Print and shaded views of the part. All mm, measured from the part's lowest x, y and z. A direction names the side the tool comes from. Round coordinates to 2 decimals unless told otherwise and drop trailing zeros. Write each loop counter-clockwise with the first axis right and the second up, starting at its lowest first coordinate (ties: lowest second). Pieces come first, ordered by that corner, then holes. Notation, with made-up numbers: M -34,-26 L -28,-26 A8 cw -28,-17 Z; hole C 16.25,-38 d8. An arc over 180 degrees is marked long. Write item = value, one per line.
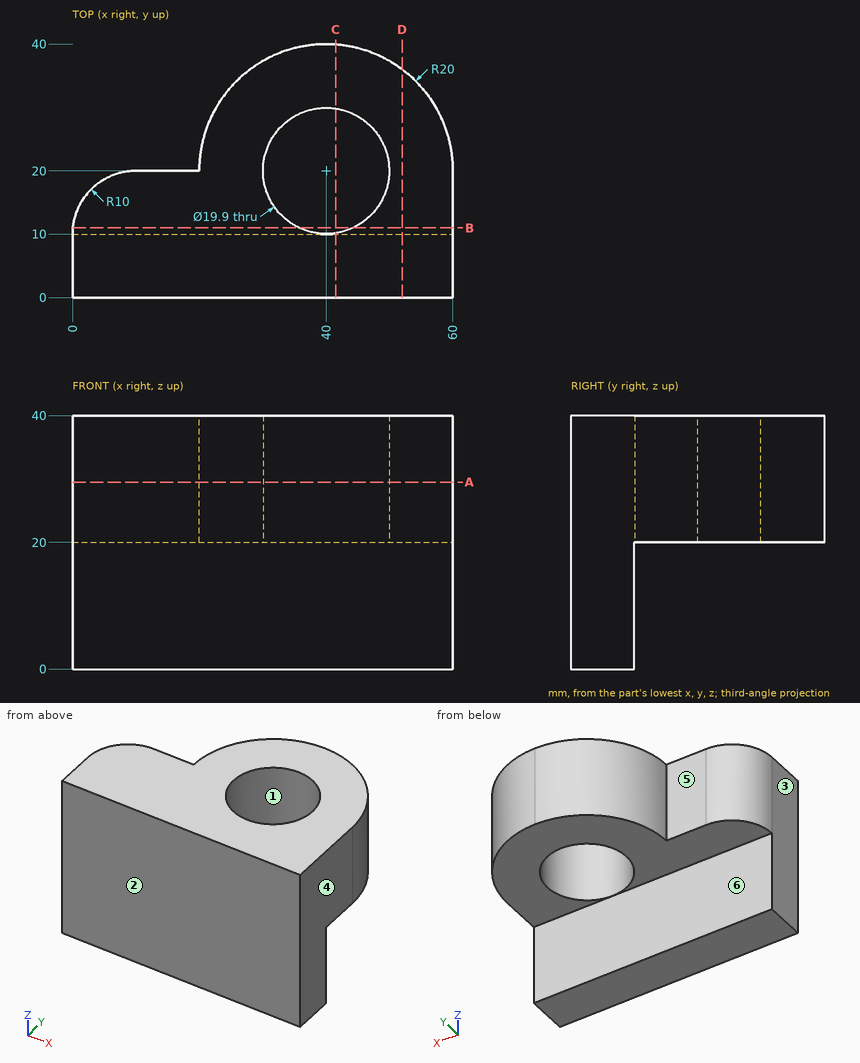
1. Tool access for the marked faces 4, 5 and 6: list every direction of +Z, -Z, +X, -X, +Y, -Y with a clear straight run to the whole face (end or side of a thin tool).
Responses:
face_4 = +Z, -Z, +X, +Y, -Y
face_5 = +Z, -Z, -X, +Y
face_6 = -Z, +X, -X, +Y
2. Band-saw the part on D-D (x = 52). List the corners of the cut face in (y, z), plus the area to 3 significant figures.
Responses:
outline = M 0,0 L 10,0 L 10,20 L 36,20 L 36,40 L 0,40 Z
area = 920 mm²
3. Band-saw the part on B-B (y = 11). List the corners of the cut face in (x, z).
Responses:
outline = M 0.05,20 L 35.76,20 L 35.76,40 L 0.05,40 Z; M 44.24,20 L 60,20 L 60,40 L 44.24,40 Z
4. Band-saw the part on A-A (z = 29.5). List the corners of the cut face in (x, y), plus the area to 3 significant figures.
Responses:
outline = M 0,0 L 60,0 L 60,20 A20 ccw 20,20 L 10,20 A10 ccw 0,10 Z; hole C 40,20 d19.9
area = 1,500 mm²
5. Band-saw the part on C-C (x = 41.5). List the corners of the cut face in (y, z), plus the area to 3 significant figures.
Responses:
outline = M 0,0 L 10,0 L 10,20 L 10.16,20 L 10.16,40 L 0,40 Z; M 29.84,20 L 39.94,20 L 39.94,40 L 29.84,40 Z
area = 605 mm²
6. Mould opens along X. For the marked faces 1, 2 and 3 say: pulls with the +X half, pulls with the -X half, needs draft (parallel to the pull), parting line crosses it, or undercut.
Responses:
face_1 = undercut
face_2 = needs draft
face_3 = pulls with the -X half
7. Flat gauge pins, fed straight in: pin 1 (6 mm diameter, centred on y = 34, z = 19.5, fed in from +X); pin 2 (6 mm diameter, centred on x = 42.5, z = 7.5, fed in from +Y); pin 3 (11 mm diameter, centred on x = 12.5, z = 25.5, fed in from +Y). Where does each tip first touch, or does it go through?
Responses:
pin_1 = 56.68
pin_2 = 10
pin_3 = 20
8. Probe probe 1 along Y at (x, z) = (45, 12); probe 2 along Z at (x, y) = (18, 11.5); probe 3 along Y at (x, z) = (19, 35). List the from-to ranges inside material, lowest first.
Responses:
probe_1 = 0 to 10
probe_2 = 20 to 40
probe_3 = 0 to 20
